The listing builds one solid part. Answer for the finished solid, in the listing's coordinates (mm). A direction names the side the tool comes from. Coordinates: 2 decimals unless noted, no trailing zeros. Order: outer loops, then holes, each group sorted by start corner. A loop starts at its lowest first (then second) coordinate and runs counter-clockwise, first axis right, second up. Notation, with made-up numbers: (64.5, 12) -> (71.5, 12) arc R20 cw to (71.5, 23) -> close; hole circle Ø1 at (5, 66). An arc over 180 degrees is marked (long way). Return JSON: item names as keys, results as strings.
from build123d import *

# Parameters (mm, degrees)
EXTRUDE_1_DEPTH = 15


with BuildPart() as part:
    # 草图1 → 拉伸-薄壁1 (new, symmetric)
    with BuildSketch(Plane(origin=(-54.389817032, 234.459616021, 1948), x_dir=(0, 0, 1), z_dir=(0, -1, 0))):
        with BuildLine():
            Line((-669.781125, 73.589656521), (-691.82105475, 115.041248428))
            ThreePointArc((-691.82105475, 115.041248428), (-745.5, 147.295), (-799.17894525, 115.041248428))
            Line((-799.17894525, 115.041248428), (-821.218875, 73.589656521))
            ThreePointArc((-821.218875, 73.589656521), (-831.170890239, 63.02817405), (-845.113030011, 59.002722785))
            Line((-845.113030011, 59.002722785), (-1396.721100985, 51.239926214))
            ThreePointArc((-1396.721100985, 51.239926214), (-1447.243731538, -0.360559418), (-1396, -51.245))
            Line((-1396, -51.245), (0, -51.245))
            ThreePointArc((0, -51.245), (51.244076889, -0.307585387), (0.615159693, 51.24130759))
            Line((0.615159693, 51.24130759), (-645.830117895, 59.001981486))
            ThreePointArc((-645.830117895, 59.001981486), (-659.804837816, 63.013373698), (-669.781125, 73.589656521))
        make_face()
        with BuildLine():
            Line((-673.7544, 71.477054861), (-695.79432975, 112.928646768))
            ThreePointArc((-695.79432975, 112.928646768), (-745.5, 142.795), (-795.20567025, 112.928646768))
            Line((-795.20567025, 112.928646768), (-817.2456, 71.477054861))
            ThreePointArc((-817.2456, 71.477054861), (-828.826126823, 59.187329803), (-845.049707649, 54.503168332))
            Line((-845.049707649, 54.503168332), (-1396.657778624, 46.74037176))
            ThreePointArc((-1396.657778624, 46.74037176), (-1442.743842926, -0.328897453), (-1396, -46.745))
            Line((-1396, -46.745), (0, -46.745))
            ThreePointArc((0, -46.745), (46.744157951, -0.280575254), (0.561140401, 46.741631833))
            Line((0.561140401, 46.741631833), (-645.884137187, 54.50230573))
            ThreePointArc((-645.884137187, 54.50230573), (-662.145629459, 59.170107576), (-673.7544, 71.477054861))
        make_face(mode=Mode.SUBTRACT)
    extrude(amount=EXTRUDE_1_DEPTH, both=True)


solid = part.part
1. The part is cut by section B-B on x = -89. Give the vertices of the cut face in (y, z).
Answer block:
{"outline": "(219.46, 514.21) -> (249.46, 514.21) -> (249.46, 520.58) -> (219.46, 520.58) -> close; (219.46, 1979.42) -> (249.46, 1979.42) -> (249.46, 1985.79) -> (219.46, 1985.79) -> close"}
2. The part is cut by section A-A on y = 231.25. Give the vertices of the cut face in (x, z) (3 decimals).
Answer block:
{"outline": "(-169.431, 1148.821) -> (-127.979, 1126.781) arc R27.5 cw to (-113.393, 1102.887) -> (-105.63, 551.279) arc R51.245 ccw to (-3.145, 552) -> (-3.145, 1948) arc R51.245 ccw to (-105.631, 1948.615) -> (-113.392, 1302.17) arc R27.5 cw to (-127.979, 1278.219) -> (-169.431, 1256.179) arc R60.795 ccw to start; hole (-167.318, 1152.794) -> (-125.867, 1130.754) arc R32 cw to (-108.893, 1102.95) -> (-101.13, 551.342) arc R46.745 ccw to (-7.645, 552) -> (-7.645, 1948) arc R46.745 ccw to (-101.131, 1948.561) -> (-108.892, 1302.116) arc R32 cw to (-125.867, 1274.246) -> (-167.318, 1252.206) arc R56.295 ccw to start"}
3. Each of these flat-tipped pins is pushed along its axis until it touches: pin 1 Ø1.5 at (x, y) = (-129.5, 230.5) entering from +Z; pin 2 Ø1.5 at (x, y) = (-151.5, 230.5) entering from +Z; pin 3 Ø12 at (x, y) = (-159.5, 237.5) entering from -Z. Where does it stop, or does it pass through?
Answer block:
{"pin 1": "stops at z = 1277.81", "pin 2": "stops at z = 1266.11", "pin 3": "stops at z = 1140.35"}
4. For faces 1 (the face through (-53.085, 234.25, 1994.727)), 2 (the face through (-149, 234.25, 1137.96)), determine the directions among +Z, -Z, +X, -X, +Y, -Y from which every point of the face is accessible in a straight line to the end or side of a thin tool.
Answer block:
{"face 1": "+Y, -Y", "face 2": "-Z, -X, +Y, -Y"}
5. Consider line 1 (X direction, y = 238.75, z = 1312.5); line 2 (X direction, y = 231.5, z = 1585.5); line 3 (Z direction, x = -31.5, y = 237.25). Determine where each line is inside the solid, lowest interval first. Write a range as from..to.
Answer block:
{"line 1": "x = -113.27..-108.77, -7.64..-3.14", "line 2": "x = -109.99..-105.49, -7.64..-3.14", "line 3": "z = 506.15..511.24, 1988.76..1993.85"}
6. Determine the mould class of faces 3 (the face through (-201.678, 234.25, 1203.421)), 4 (the face through (-55.15, 234.25, 500.76)), 5 (the face through (-113.436, 234.25, 1286.06)) for opening direction X: pulls with the +X half, pulls with the -X half, needs draft (parallel to the pull), parting line crosses it, or undercut.
Answer block:
{"face 3": "pulls with the -X half", "face 4": "parting line crosses it", "face 5": "undercut"}
7. The part is cut by section C-C on z = 1491.5. Give the vertices of the cut face in (x, y).
Answer block:
{"outline": "(-111.12, 219.46) -> (-106.62, 219.46) -> (-106.62, 249.46) -> (-111.12, 249.46) -> close; (-7.64, 219.46) -> (-3.14, 219.46) -> (-3.14, 249.46) -> (-7.64, 249.46) -> close"}
